```python
from build123d import *


with BuildPart() as part:
    # Sketch1 → Revolve1 (revolve)
    with BuildSketch(Plane.XY, mode=Mode.PRIVATE) as revolve1_sk:
        Polygon((1542.193616015, 1896.149332348), (1541.965999426, 1896.149332348), (1541.852191131, 1896.035524053), (1541.852191131, 1894.100783041), (1542.07980772, 1893.873166452), (1545.038823386, 1893.873166452), (1545.266439975, 1894.100783041), (1545.266439975, 1894.726728663), (1544.981919238, 1895.0112494), (1542.990274079, 1895.0112494), (1542.990274079, 1894.897441105), (1542.193616015, 1894.897441105), align=None)
        Polygon((1542.990274079, 1895.295770137), (1542.990274079, 1895.0112494), (1544.981919238, 1895.0112494), (1544.697398501, 1895.295770137), align=None)
    revolve(revolve1_sk.sketch.rotate(Axis((1539.352588353, 1902.873166452, 0), (1, 0, 0)), 270), axis=Axis((1539.352588353, 1902.873166452, 0), (1, 0, 0)))


solid = part.part
```
Geometry: final body of the model. Coordinates: model frame, mm. A direction names the side the tool comes from. Round coordinates to 2 decimals unless told otherwise and drop trailing zeros. Loops run counter-clockwise (first coordinate to the right, second up) from the corner with the lowest first, then second, coordinate; pieces in that order, holes last.
Item 1: Reachability of faces 1 (the flat face through (1541.852, 1908, 5)), 2 (the cylindrical face through (1542.586, 1897.483, -5.878)) from +Z, -Z, +X, -X, +Y, -Y: full face, straight path, thin tool, end or side. Return the list, or none.
Checked values:
face 1: +Z, -Z, -X, +Y, -Y
face 2: none
Item 2: Contact query for flat-ended pins moving along their axis: P1, Ø1, axis at x = 1543, z = 0.5, coming from the +Y side; P2, Ø8, axis at y = 1903.5, z = -2.5, coming from the -X side; P3, Ø2, axis at x = 1544, z = 5.5, coming from the +Y side; P4, Ø1.5, axis at x = 1542.5, z = 5.5, coming from the +Y side. Output: stop coordinate, or through.
Checked values:
P1: stops at y = 1911.87
P2: passes through
P3: stops at y = 1910.67
P4: stops at y = 1910.52
Item 3: Mould query, pull axis X, two halves, no side actions, for faces 3 (the cylindrical face through (1543.83, 1910.27, -1.64)), 4 (the flat face through (1542.99, 1910, -3)), 5 (the flat face through (1545.266, 1909, 6)). Classes: released by +X, released by -X, zero draft, split by the parting line, or undercut.
Checked values:
face 3: zero draft
face 4: undercut
face 5: released by +X
Item 4: Line query: L1, parallel to Z at x = 1542.85, y = 1902.75; L2, parallel to Y at x = 1542.7, z = 0; L3, parallel to Z at x = 1544.1, y = 1908.25. Output: solid intervals per line, ascending.
Checked values:
L1: z = -9 to -7.97, 7.97 to 9
L2: y = 1893.87 to 1894.9, 1910.85 to 1911.87
L3: z = -7.22 to -5.34, 5.34 to 7.22
Item 5: Section B-B, the plane x = 1544.05. Output: boundary loops of the cut face in (y, z), plus the area to 3 significant figures.
Checked values:
outline: circle Ø18 at (1902.87, 0); hole circle Ø15.15 at (1902.87, 0)
area: 74.1 mm2
Item 6: Section A-A, the plane z = 0. Output: boundary loops of the cut face in (x, y), plus the area to 3 significant figures.
Checked values:
outline: (1541.85, 1894.1) - (1542.08, 1893.87) - (1545.04, 1893.87) - (1545.27, 1894.1) - (1545.27, 1894.73) - (1544.7, 1895.3) - (1542.99, 1895.3) - (1542.99, 1894.9) - (1542.19, 1894.9) - (1542.19, 1896.15) - (1541.97, 1896.15) - (1541.85, 1896.04) - close; (1541.85, 1909.71) - (1541.97, 1909.6) - (1542.19, 1909.6) - (1542.19, 1910.85) - (1542.99, 1910.85) - (1542.99, 1910.45) - (1544.7, 1910.45) - (1545.27, 1911.02) - (1545.27, 1911.65) - (1545.04, 1911.87) - (1542.08, 1911.87) - (1541.85, 1911.65) - close
area: 9.22 mm2
